```python
from build123d import *

# Parameters (mm, degrees)
BRACKET_BODY_DEPTH            = 45
TOP_SLOT_18X72_DEPTH          = 45
PIVOT_BOSS_DEPTH              = 45
PIVOT_BORE_SKETCH_R           = 9
PIVOT_BORE_18_DEPTH           = 72
FLANGE_CORNER_FILLETS_R22_5_R = 22.5
FLANGE_HOLES_SKETCH_R         = 9
FLANGE_HOLES_2X_18_DEPTH      = 72
SIDE_HOLE_SKETCH_R            = 9
SIDE_HOLE_18_DEPTH            = 72


with BuildPart() as part:
    # Bracket Profile Sketch → Bracket Body (new, symmetric)
    with BuildSketch(Plane.XY):
        Polygon((0, 0), (0, 18), (121.5, 18), (121.5, 108), (256.5, 108), (256.5, 0), (238.5, 0), (238.5, 90), (139.5, 90), (139.5, 0), align=None)
    extrude(amount=BRACKET_BODY_DEPTH, both=True)

    # Top Slot Sketch → Top Slot 18x72 (cut, symmetric)
    with BuildSketch(Plane(origin=(0, 108, 0), x_dir=(1, 0, 0), z_dir=(0, 1, 0))):
        with BuildLine():
            Line((162, 9), (216, 9))
            ThreePointArc((216, 9), (225, 0), (216, -9))
            Line((216, -9), (162, -9))
            ThreePointArc((162, -9), (153, 0), (162, 9))
        make_face()
    extrude(amount=TOP_SLOT_18X72_DEPTH, both=True, mode=Mode.SUBTRACT)

    # Pivot Boss Sketch → Pivot Boss (add)
    with BuildSketch(Plane(origin=(0, 18, 0), x_dir=(1, 0, 0), z_dir=(0, 1, 0))):
        with BuildLine():
            Line((81, 22.5), (121.5, 22.5))
            Line((121.5, 22.5), (121.5, -22.5))
            Line((121.5, -22.5), (81, -22.5))
            ThreePointArc((81, -22.5), (58.5, 0), (81, 22.5))
        make_face()
    extrude(amount=PIVOT_BOSS_DEPTH)

    # Pivot Bore Sketch → Pivot Bore Ø18 (cut)
    with BuildSketch(Plane(origin=(0, 63, 0), x_dir=(1, 0, 0), z_dir=(0, 1, 0))):
        with Locations(Location((81, 0, 0), (0, 0, 270))):
            Circle(PIVOT_BORE_SKETCH_R)
    extrude(amount=-PIVOT_BORE_18_DEPTH, mode=Mode.SUBTRACT)

    # Flange Corner Fillets R22.5
    flange_corner_fillets_r22_5_edges = [part.edges().sort_by_distance(p)[0] for p in [
        (0, 9, -45),
        (0, 9, 45),
    ]]
    fillet(flange_corner_fillets_r22_5_edges, radius=FLANGE_CORNER_FILLETS_R22_5_R)

    # Flange Holes Sketch → Flange Holes 2xØ18 (cut)
    with BuildSketch(Plane(origin=(0, 18, 0), x_dir=(1, 0, 0), z_dir=(0, 1, 0))):
        with Locations(Location((22.5, 22.5, 0), (0, 0, 270))):
            Circle(FLANGE_HOLES_SKETCH_R)
        with Locations(Location((22.5, -22.5, 0), (0, 0, 270))):
            Circle(FLANGE_HOLES_SKETCH_R)
    extrude(amount=-FLANGE_HOLES_2X_18_DEPTH, mode=Mode.SUBTRACT)

    # Side Hole Sketch → Side Hole Ø18 (cut)
    with BuildSketch(Plane(origin=(256.5, 0, 0), x_dir=(0, 0, -1), z_dir=(1, 0, 0))):
        with Locations((0, 18)):
            Circle(SIDE_HOLE_SKETCH_R)
    extrude(amount=-SIDE_HOLE_18_DEPTH, mode=Mode.SUBTRACT)


solid = part.part
```
Part model, mm, in its own coordinate system. A direction names the side the tool comes from. Round coordinates to 2 decimals unless told otherwise and drop trailing zeros. Write each loop counter-clockwise with the first axis right and the second up, starting at its lowest first coordinate (ties: lowest second). Pieces come first, ordered by that corner, then holes.
Item 1: Drop flat-ended pins along their axis: pin 1 Ø10 at (y, z) = (22, 4.5) entering from +X; pin 2 Ø11 at (x, z) = (22.5, -22.5) entering from +Y; pin 3 Ø12 at (x, z) = (51, 4) entering from +Y; pin 4 Ø22.5 at (x, z) = (93, 1.5) entering from +Y. Give the stop position or say it passes through.
Results:
pin 1: stops at x = 256.5
pin 2: passes through
pin 3: stops at y = 18
pin 4: stops at y = 63
Item 2: Probe L1, parallel to Z at x = 22, y = 12; L2, parallel to X at y = 7.75, z = -22.5; L3, parallel to X at y = 42, z = 0. List the from-to ranges inside material, lowest first.
Results:
L1: z = -44.99 to -31.49, -13.51 to 13.51, 31.49 to 44.99
L2: x = 0 to 13.5, 31.5 to 139.5, 238.5 to 256.5
L3: x = 58.5 to 72, 90 to 139.5, 238.5 to 256.5
Item 3: Two-plate mould, pull along X, no slides. Class faces 5 (the flat face through (139.5, 46, 1)), 6 (the flat face through (101, 40, -22.5)), 7 (the cylindrical face through (58.505, 40.185, 0.495)): +X half, -X half, draft (parallel to the pull), parting line (faces both ways), or undercut.
Results:
face 5: undercut
face 6: draft
face 7: -X half
Item 4: Which spindle directions (+Z, -Z, +X, -X, +Y, -Y) get a long thin tool onto all of the face, cutting with end or side? Do faces 1 (the flat face through (189, 99, 9)), 2 (the flat face through (90.4, 63, -0.3)), 3 (the flat face through (102, 40, 22.5)), 4 (the flat face through (46, 18, 1)). Say none if no direction does.
Results:
face 1: +Y, -Y
face 2: +Z, -Z, -X, +Y
face 3: +Z, -X, +Y
face 4: -X, +Y
Item 5: Cut at A-A, the plane y = 52. Give the cut face in (x, z).
Results:
outline: (81, -22.5) - (121.5, -22.5) - (121.5, -45) - (139.5, -45) - (139.5, 45) - (121.5, 45) - (121.5, 22.5) - (81, 22.5) arc R22.5 ccw to start; (238.5, -45) - (256.5, -45) - (256.5, 45) - (238.5, 45) - close; hole circle Ø18 at (81, 0)
Item 6: Cut at D-D, the plane x = 179.5. Give the cut face in (y, z), plus the area to 3 significant figures.
Results:
outline: (90, -45) - (108, -45) - (108, -9) - (90, -9) - close; (90, 9) - (108, 9) - (108, 45) - (90, 45) - close
area: 1,300 mm2
Item 7: Cut at C-C, the plane y = 77. Give the cut face in (x, z).
Results:
outline: (121.5, -45) - (139.5, -45) - (139.5, 45) - (121.5, 45) - close; (238.5, -45) - (256.5, -45) - (256.5, 45) - (238.5, 45) - close
Item 8: Cut at B-B, the plane z = 0. Give the cut face in (x, y).
Results:
outline: (0, 0) - (72, 0) - (72, 63) - (58.5, 63) - (58.5, 18) - (0, 18) - close; (90, 0) - (139.5, 0) - (139.5, 90) - (153, 90) - (153, 108) - (121.5, 108) - (121.5, 63) - (90, 63) - close; (225, 90) - (238.5, 90) - (238.5, 27) - (256.5, 27) - (256.5, 108) - (225, 108) - close; (238.5, 0) - (256.5, 0) - (256.5, 9) - (238.5, 9) - close
